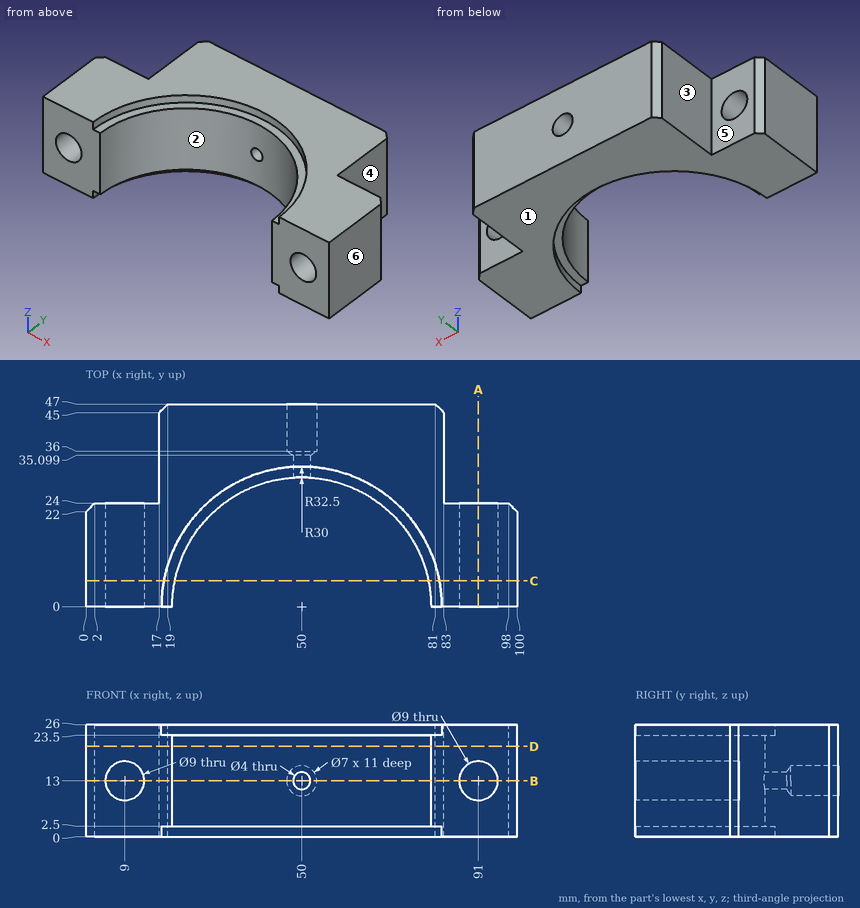
Verification items for this drawing (mm, ordinates from the low corner). A direction names the side the tool comes from. Give positions to 0.01 mm unless a question says otherwise; leave off trailing zeros. Loops run counter-clockwise (first coordinate to the right, second up) from the corner with the lowest first, then second, coordinate; pieces in that order, holes last. Notation, with made-up numbers: (-7, 1.5) - (41, 1.5) arc R13 ccw to (41, 11.5) - close; hole circle Ø2 at (-34.75, 6.5). An arc over 180 degrees is marked (long way). Write item = value, one per line. Start each with the question number.
Q1. Cross-section at A-A, the plane x = 91. Enter the section's corners in (y, z), and give its area (3 significant figures).
Q2. Mould release check, pull along X, two halves, no side actions. Record for the marked faces 1, 2 and 3: released by +X, released by -X, zero draft, split by the parting line, or undercut.
Q3. Cross-section at B-B, the plane z = 13. State how many separate pieces and enclosed holes the cut face has, and give its area (3 significant figures).
Q4. Thickness scan on line 1 (X direction, y = 20.5, z = 12.5); line 2 (Z direction, x = 50, y = 32.1); line 3 (Y direction, x = 10.5, z = 3.75). Record the ranges inside material, lowest first.
Q5. Tool access check on the marked faces 4, 5 and 6. Record the directions out of +Z, -Z, +X, -X, +Y, -Y that give a thin tool (end or side, any length) a straight path to the whole face; none if there is none.
Q6. Depth check by flat-ended pin: P1, Ø1.5, axis at y = 21.5, z = 11.5, coming from the -X side; P2, Ø14.5, axis at x = 9, z = 13, coming from the +Y side; P3, Ø10.5, axis at y = 36.5, z = 16, coming from the +X side; P4, Ø10, axis at y = 40, z = 22, coming from the -X side. Enter the tip coordinate at first touch or a pass-through.
Q7. Cross-section at D-D, the plane z = 21. Enter the section's corners in (x, y).
Q8. Cross-section at C-C, the plane y = 6. Enter the section's corners in (x, z), and give its area (3 significant figures).
Answer key:
q1.outline = (0, 0) - (24, 0) - (24, 8.5) - (0, 8.5) - close; (0, 17.5) - (24, 17.5) - (24, 26) - (0, 26) - close
q1.area = 408 mm^2
q2.face_1 = zero draft
q2.face_2 = undercut
q2.face_3 = released by -X
q3.separate_pieces = 4
q3.enclosed_holes = 0
q3.area = 1,960 mm^2
q4.line_1 = 0 to 4.53, 13.47 to 28.1, 71.9 to 86.53, 95.47 to 100
q4.line_2 = 2.5 to 11, 15 to 23.5
q4.line_3 = 0 to 24
q5.face_4 = +Z, -Z, +X, +Y
q5.face_5 = +Z, -Z, -X, +Y
q5.face_6 = +Z, -Z, +X, +Y, -Y
q6.P1 = 0
q6.P2 = 24
q6.P3 = 83
q6.P4 = 17
q7.outline = (0, 0) - (20, 0) arc R30 cw to (80, 0) - (100, 0) - (100, 22) - (98, 24) - (83, 24) - (83, 45) - (81, 47) - (19, 47) - (17, 45) - (17, 24) - (2, 24) - (0, 22) - close
q8.outline = (0, 0) - (18.06, 0) - (18.06, 2.5) - (20.61, 2.5) - (20.61, 23.5) - (18.06, 23.5) - (18.06, 26) - (0, 26) - close; (79.39, 2.5) - (81.94, 2.5) - (81.94, 0) - (100, 0) - (100, 26) - (81.94, 26) - (81.94, 23.5) - (79.39, 23.5) - close; hole circle Ø9 at (9, 13); hole circle Ø9 at (91, 13)
q8.area = 919 mm^2
